```python
from build123d import *

# Parameters (mm, degrees)
SKETCH_1_W          = 20
SKETCH_1_H          = 300
EXTRUDE_1_DEPTH     = 330
SKETCH_2_W          = 580
SKETCH_2_H          = 240
CUT_EXTRUDE_1_DEPTH = 364.042697213
FILLET_1_R          = 60


with BuildPart() as part:
    # 草图1 → 凸台-拉伸1 (new, symmetric)
    with BuildSketch(Plane.XY):
        Rectangle(SKETCH_1_W, SKETCH_1_H)
    extrude(amount=EXTRUDE_1_DEPTH, both=True)

    # 草图2 → 切除-拉伸1 (cut, through all)
    with BuildSketch(Plane(origin=(10, 0, 0), x_dir=(0, 0, -1), z_dir=(1, 0, 0))):
        with Locations((40, -30)):
            Rectangle(SKETCH_2_W, SKETCH_2_H)
    extrude(amount=-CUT_EXTRUDE_1_DEPTH, mode=Mode.SUBTRACT)

    # 圆角1
    fillet_1_edges = [part.edges().sort_by_distance(p)[0] for p in [
        (0, 90, 250),
    ]]
    fillet(fillet_1_edges, radius=FILLET_1_R)


solid = part.part
```
Read the model definition and answer for the solid it produces. Units are mm, in the model's axes. A direction names the side the tool comes from. Coordinates: 2 decimals unless noted, no trailing zeros. Loops run counter-clockwise (first coordinate to the right, second up) from the corner with the lowest first, then second, coordinate; pieces in that order, holes last.
(1) The part is cut by section A-A (x = 0.25). Determine the outline of the cut face in (y, z), and give its area (3 significant figures).
Solution:
outline: (-150, 250) - (30, 250) arc R60 cw to (90, 190) - (90, -330) - (150, -330) - (150, 330) - (-150, 330) - close
area: 59,600 mm2
(2) Flat-ended cylindrical pins translate along their axes: pin 1 Ø6 at (x, y) = (1.5, -81) entering from -Z; pin 2 Ø12 at (x, z) = (-4, 92.5) entering from -Y. Find the tip coordinate at first contact, or state that the pin passes through.
Solution:
pin 1: stops at z = 250
pin 2: stops at y = 90
(3) The part is cut by section B-B (z = -214.5). Determine the outline of the cut face in (x, y).
Solution:
outline: (-10, 90) - (10, 90) - (10, 150) - (-10, 150) - close
(4) Consider line 1 along Z through (x, y) = (-8.5, -136.5); line 2 along Y through (x, z) = (-5.5, 66); line 3 along Y through (x, z) = (-1.5, 222.5). Determine where each line is inside the solid, lowest interval first.
Solution:
line 1: z = 250 to 330
line 2: y = 90 to 150
line 3: y = 80.44 to 150
(5) The part is cut by section C-C (y = -114.5). Determine the outline of the cut face in (x, z), and give its area (3 significant figures).
Solution:
outline: (-10, 250) - (10, 250) - (10, 330) - (-10, 330) - close
area: 1,600 mm2
(6) A tool of negligible diameter and unlimited length cuts with its end or side. For faces 1 (the face through (0, 2, 330)), 2 (the face through (0, -61, 250)), from which of +Z, -Z, +X, -X, +Y, -Y can it reach the whole face along a straight path? Write none if from no direction.
Solution:
face 1: +Z, +X, -X, +Y, -Y
face 2: -Z, +X, -X, -Y
